```python
from build123d import *

# Parameters (mm, degrees)
SKETCH1_R           = 5
BOSS_EXTRUDE1_DEPTH = 2
SKETCH2_R           = 3.5
BOSS_EXTRUDE2_DEPTH = 5.4
SKETCH3_R           = 8.5
BOSS_EXTRUDE3_DEPTH = 1.5
SKETCH4_R           = 3.5
BOSS_EXTRUDE4_DEPTH = 18
SKETCH5_R           = 8.5
BOSS_EXTRUDE5_DEPTH = 1.5
SKETCH6_R           = 3.5
BOSS_EXTRUDE6_DEPTH = 5.4
SKETCH7_R           = 2.885
BOSS_EXTRUDE7_DEPTH = 6.57


with BuildPart() as part:
    # Sketch1 → Boss-Extrude1 (new body)
    with BuildSketch(Plane(origin=(0, 0, 0), x_dir=(1, 0, 0), z_dir=(0, 1, 0))):
        with Locations(Location((0, 0, 0), (0, 0, 270))):
            Circle(SKETCH1_R)
    extrude(amount=BOSS_EXTRUDE1_DEPTH)

    # Sketch2 → Boss-Extrude2 (add)
    with BuildSketch(Plane(origin=(0, 2, 0), x_dir=(1, 0, 0), z_dir=(0, 1, 0))):
        with Locations(Location((0, 0, 0), (0, 0, 90))):
            Circle(SKETCH2_R)
    extrude(amount=BOSS_EXTRUDE2_DEPTH)

    # Sketch3 → Boss-Extrude3 (add)
    with BuildSketch(Plane(origin=(0, 7.4, 0), x_dir=(1, 0, 0), z_dir=(0, 1, 0))):
        with Locations(Location((0, 0, 0), (0, 0, 270))):
            Circle(SKETCH3_R)
    extrude(amount=BOSS_EXTRUDE3_DEPTH)

    # Sketch4 → Boss-Extrude4 (add)
    with BuildSketch(Plane(origin=(0, 8.9, 0), x_dir=(1, 0, 0), z_dir=(0, 1, 0))):
        with Locations(Location((0, 0, 0), (0, 0, 90))):
            Circle(SKETCH4_R)
    extrude(amount=BOSS_EXTRUDE4_DEPTH)

    # Sketch5 → Boss-Extrude5 (add)
    with BuildSketch(Plane(origin=(0, 26.9, 0), x_dir=(1, 0, 0), z_dir=(0, 1, 0))):
        with Locations(Location((0, 0, 0), (0, 0, 270))):
            Circle(SKETCH5_R)
    extrude(amount=BOSS_EXTRUDE5_DEPTH)

    # Sketch6 → Boss-Extrude6 (add)
    with BuildSketch(Plane(origin=(0, 28.4, 0), x_dir=(1, 0, 0), z_dir=(0, 1, 0))):
        with Locations(Location((0, 0, 0), (0, 0, 90))):
            Circle(SKETCH6_R)
    extrude(amount=BOSS_EXTRUDE6_DEPTH)

    # Sketch7 → Boss-Extrude7 (add)
    with BuildSketch(Plane(origin=(0, 33.8, 0), x_dir=(1, 0, 0), z_dir=(0, 1, 0))):
        with Locations(Location((0, 0, 0), (0, 0, 270))):
            Circle(SKETCH7_R)
    extrude(amount=BOSS_EXTRUDE7_DEPTH)


solid = part.part
```
Part model, mm, in its own coordinate system. A direction names the side the tool comes from. Give positions to 0.01 mm unless a question says otherwise; leave off trailing zeros. Order: outer loops, then holes, each group sorted by start corner. A loop starts at its lowest first (then second) coordinate and runs counter-clockwise, first axis right, second up. Notation, with made-up numbers: (69.25, 74) - (121.25, 74) arc R31 ccw to (121.25, 107) - close; hole circle Ø8 at (86.5, 73.5). An arc over 180 degrees is marked (long way). Use one line per item in the form item = value.
Item 1: Which spindle directions (+Z, -Z, +X, -X, +Y, -Y) get a long thin tool onto all of the face, cutting with end or side? Do faces 1 (the face through (-4.88, 0.99, -1.08)), 2 (the face through (0, 8.9, 4)), 3 (the face through (0, 40.37, 0)), 4 (the face through (3.417, 31.062, 0.759)). Say none if no direction does.
Solution:
face_1 = -Y
face_2 = none
face_3 = +Z, -Z, +X, -X, +Y
face_4 = +Y
Item 2: Slice it at D-D on x = 0. Give the cut face in (y, z) (3 decimals), and give its area (3 significant figures).
Solution:
outline = (0, -5) - (2, -5) - (2, -3.5) - (7.4, -3.5) - (7.4, -8.5) - (8.9, -8.5) - (8.9, -3.5) - (26.9, -3.5) - (26.9, -8.5) - (28.4, -8.5) - (28.4, -3.5) - (33.8, -3.5) - (33.8, -2.885) - (40.37, -2.885) - (40.37, 2.885) - (33.8, 2.885) - (33.8, 3.5) - (28.4, 3.5) - (28.4, 8.5) - (26.9, 8.5) - (26.9, 3.5) - (8.9, 3.5) - (8.9, 8.5) - (7.4, 8.5) - (7.4, 3.5) - (2, 3.5) - (2, 5) - (0, 5) - close
area = 311 mm2
Item 3: Slice it at B-B on x = 6. Give the cut face in (y, z).
Solution:
outline = (7.4, -6.02) - (8.9, -6.02) - (8.9, 6.02) - (7.4, 6.02) - close; (26.9, -6.02) - (28.4, -6.02) - (28.4, 6.02) - (26.9, 6.02) - close
Item 4: Pin check, flat tips, straight feed: pin 1 Ø6 at (x, z) = (0, -4.5) entering from -Y; pin 2 Ø1 at (y, z) = (23, 0) entering from -X; pin 3 Ø4 at (x, z) = (4, 4) entering from +Y; pin 4 Ø6 at (y, z) = (35.5, 4) entering from +X. Stop position of each tip, or through.
Solution:
pin_1 = 0
pin_2 = -3.5
pin_3 = 28.4
pin_4 = 3.15
Item 5: Probe probe 1 along Y at (x, z) = (-3.5, -3.5); probe 2 along Y at (x, z) = (-7.5, 2.25); probe 3 along X at (y, z) = (22, 0). List the from-to ranges inside material, lowest first. Write a range as from..to.
Solution:
probe_1 = 0..2, 7.4..8.9, 26.9..28.4
probe_2 = 7.4..8.9, 26.9..28.4
probe_3 = -3.5..3.5
Item 6: Slice it at C-C on z = 0. Give the cut face in (x, y) (3 decimals), and give its area (3 significant figures).
Solution:
outline = (-8.5, 7.4) - (-3.5, 7.4) - (-3.5, 2) - (-5, 2) - (-5, 0) - (5, 0) - (5, 2) - (3.5, 2) - (3.5, 7.4) - (8.5, 7.4) - (8.5, 8.9) - (3.5, 8.9) - (3.5, 26.9) - (8.5, 26.9) - (8.5, 28.4) - (3.5, 28.4) - (3.5, 33.8) - (2.885, 33.8) - (2.885, 40.37) - (-2.885, 40.37) - (-2.885, 33.8) - (-3.5, 33.8) - (-3.5, 28.4) - (-8.5, 28.4) - (-8.5, 26.9) - (-3.5, 26.9) - (-3.5, 8.9) - (-8.5, 8.9) - close
area = 311 mm2
Item 7: Two-plate mould, pull along Y, no slides. Class faces 5 (the face through (0, 0, 0)), 6 (the face through (8.428, 8.14, -1.107)), 7 (the face through (3.417, 4.662, 0.759)): released by +Y, released by -Y, zero draft, split by the parting line, or undercut.
Solution:
face_5 = released by -Y
face_6 = zero draft
face_7 = undercut
Item 8: Slice it at A-A on z = -6. Give the cut face in (x, y), and give its area (3 significant figures).
Solution:
outline = (-6.02, 7.4) - (6.02, 7.4) - (6.02, 8.9) - (-6.02, 8.9) - close; (-6.02, 26.9) - (6.02, 26.9) - (6.02, 28.4) - (-6.02, 28.4) - close
area = 36.1 mm2
